Can you work these out from the model? Positions are in its coordinate system, mm. Coordinates: 2 decimals unless noted, no trailing zeros. Order: outer loops, then holes, each group sorted by start corner. A loop starts at its lowest first (then second) coordinate and runs counter-clockwise, first axis right, second up. Notation, with made-up numbers: (26, 51.5) -> (65, 51.5) arc R16 cw to (65, 71.5) -> close; hole circle Ø7 at (78, 52). An arc over 180 degrees is marked (long way). Answer in a Markdown table with one row per item.
```python
from build123d import *

# Parameters (mm, degrees)
SKETCH1_R           = 5.5
BOSS_EXTRUDE1_DEPTH = 6


with BuildPart() as part:
    # Sketch1 → Boss-Extrude1 (new body)
    with BuildSketch(Plane.XY.offset(3)):
        Polygon((102.5, -10), (102.5, 10), (97.5, 15), (-102.5, 15), (-102.5, -15), (97.5, -15), align=None)
        with Locations(Location((-87.5, 0, 0), (0, 0, 180))):
            Circle(SKETCH1_R, mode=Mode.SUBTRACT)
        with Locations(Location((-47.5, 0, 0), (0, 0, 180))):
            Circle(SKETCH1_R, mode=Mode.SUBTRACT)
    extrude(amount=-BOSS_EXTRUDE1_DEPTH)


solid = part.part
```
(1) I need wall thicknesses on line 1 (X direction, y = 0.5, z = 1.85); line 2 (Y direction, x = -87.5, z = -0.8); line 3 (X direction, y = 3, z = -0.2). Which ranges of each line are inside material? Lowest first, please. Write a range as [from, to].
Response values:
| item | result |
|---|---|
| line 1 | [-102.5, -92.98], [-82.02, -52.98], [-42.02, 102.5] |
| line 2 | [-15, -5.5], [5.5, 15] |
| line 3 | [-102.5, -92.11], [-82.89, -52.11], [-42.89, 102.5] |
(2) We'd pull the mould along X, two halves only. Please class faces 1 (the cylindrical face through (-82, 0, 0)), 2 (the flat face through (-1, 0, 3)), 3 (the flat face through (100, 12.5, 0)): +X half, -X half, draft (parallel to the pull), parting line (faces both ways), or undercut.
Response values:
| item | result |
|---|---|
| face 1 | undercut |
| face 2 | draft |
| face 3 | +X half |
(3) Suppose I cut it at C-C (z = 1.05). Please give me the cut outline in (x, y), and give its area (3 significant figures).
Response values:
| item | result |
|---|---|
| outline | (-102.5, -15) -> (97.5, -15) -> (102.5, -10) -> (102.5, 10) -> (97.5, 15) -> (-102.5, 15) -> close; hole circle Ø11 at (-87.5, 0); hole circle Ø11 at (-47.5, 0) |
| area | 5,930 mm2 |
(4) Suppose I cut it at A-A (x = -87.5). Please give me the cut outline in (y, z).
Response values:
| item | result |
|---|---|
| outline | (-15, -3) -> (-5.5, -3) -> (-5.5, 3) -> (-15, 3) -> close; (5.5, -3) -> (15, -3) -> (15, 3) -> (5.5, 3) -> close |
(5) Suppose I cut it at B-B (y = 0). Please give me the cut outline in (x, z).
Response values:
| item | result |
|---|---|
| outline | (-102.5, -3) -> (-93, -3) -> (-93, 3) -> (-102.5, 3) -> close; (-82, -3) -> (-53, -3) -> (-53, 3) -> (-82, 3) -> close; (-42, -3) -> (102.5, -3) -> (102.5, 3) -> (-42, 3) -> close |
